CAD build for the part. Positions are in the model's coordinates, mm. Face numbers are marked on the shaded views. A direction names the side the tool comes from. Give positions to 0.01 mm unless a question says otherwise; leave off trailing zeros. Order: outer loops, then holes, each group sorted by start corner. A loop starts at its lowest first (then second) coordinate and runs counter-clockwise, first axis right, second up. Notation, with made-up numbers: M 71,24 L 110,24 A17 ccw 110,31 Z; hole C 19,-6 d9. An arc over 180 degrees is marked long. Put each result on its own line as item: value. Start each with the question number.
1) Drill centre lines: line 1 (Y direction, x = 0, z = -19.5); line 2 (X direction, y = 5, z = -25); line 3 (Z direction, x = 0.5, y = -172.5). Where is each one in solid material? Low to high. Write a range as [from, to].
2) Pin check, flat tips, straight feed: pin 1 (10 mm diameter, centred on x = 2.5, z = -7, fed in from +Y); pin 2 (4 mm diameter, centred on x = 2, y = -141, fed in from -Z). Stop position of each tip, or through.
3) Cut at C-C (z = 18). Write the cut outline in (x, y), and give its area (3 significant figures).
4) Cut at B-B (x = -11). Write the cut outline in (y, z).
5) Cut at A-A (z = -30). Write the cut outline in (x, y).
6) Cut at D-D (y = -171). Write the cut outline in (x, z).
7) Tool access for the marked faces 1 and 2: list every direction of +Z, -Z, +X, -X, +Y, -Y with a clear straight run to the whole face (end or side of a thin tool).
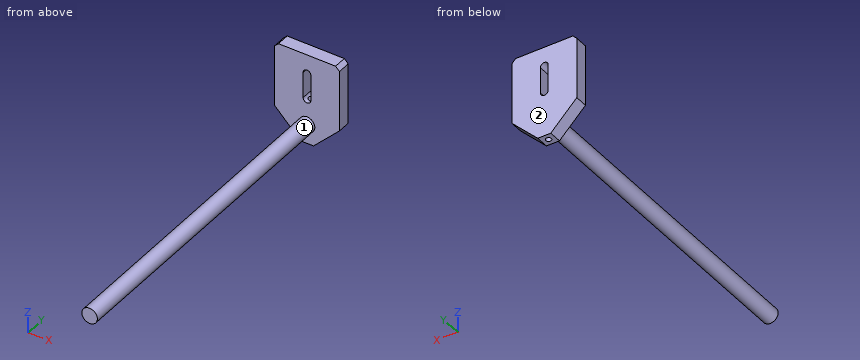
```python
from build123d import *

# Parameters (mm, degrees)
BOSS_EXTRUDE1_DEPTH   = 10
SKETCH2_R             = 6
BOSS_EXTRUDE2_DEPTH   = 260
CUT_EXTRUDE1_DEPTH    = 256.244980362
M5_TAPPED_HOLE1_D     = 4.2
M5_TAPPED_HOLE1_DEPTH = 36.9
M5_TAPPED_HOLE1_TIP   = 1.2618073
CHAMFER1_SIZE         = 3


with BuildPart() as part:
    # Sketch1 → Boss-Extrude1 (new body)
    with BuildSketch(Plane(origin=(0, 0, 0), x_dir=(1, 0, 0), z_dir=(0, 1, 0))):
        Polygon((-25, 25), (-5, 45), (5, 45), (25, 25), (25, -25), (-25, -25), align=None)
    extrude(amount=BOSS_EXTRUDE1_DEPTH)

    # Sketch2 → Boss-Extrude2 (add)
    with BuildSketch(Plane.XZ.offset(-10)):
        with Locations(Location((0, -30, 0), (0, 0, 90))):
            Circle(SKETCH2_R)
    extrude(amount=BOSS_EXTRUDE2_DEPTH)

    # Sketch3 → Cut-Extrude1 (cut, through all)
    with BuildSketch(Plane.XZ):
        with BuildLine():
            Line((-3, -10), (-3, 10))
            ThreePointArc((-3, 10), (0, 13), (3, 10))
            Line((3, 10), (3, -10))
            ThreePointArc((3, -10), (0, -13), (-3, -10))
        make_face()
    extrude(amount=-CUT_EXTRUDE1_DEPTH, mode=Mode.SUBTRACT)

    # M5 Tapped Hole1
    with Locations(Plane(origin=(0, 0, -45), x_dir=(-1, 0, 0), z_dir=(0, 0, -1))):
        with Locations((0, 5)):
            Hole(M5_TAPPED_HOLE1_D / 2, depth=M5_TAPPED_HOLE1_DEPTH)
            with Locations((0, 0, -(M5_TAPPED_HOLE1_DEPTH + M5_TAPPED_HOLE1_TIP / 2))):  # 118° drill point
                Cone(0, M5_TAPPED_HOLE1_D / 2, M5_TAPPED_HOLE1_TIP, mode=Mode.SUBTRACT)

    # Chamfer1
    chamfer1_edges = [part.edges().sort_by_distance(p)[0] for p in [
        (25, 5, 25),
        (-25, 5, 25),
    ]]
    chamfer(chamfer1_edges, length=CHAMFER1_SIZE)


solid = part.part
```
Solution:
1. line 1: [0, 2.9], [7.1, 10]
1. line 2: [-25, -2.1], [2.1, 25]
1. line 3: [-35.98, -24.02]
2. pin 1: y = 10
2. pin 2: z = -36
3. outline: M -25,0 L 25,0 L 25,10 L -25,10 Z
3. area: 500 mm²
4. outline: M 0,-39 L 10,-39 L 10,25 L 0,25 Z
5. outline: M -20,0 L -6,0 L -6,-250 L 6,-250 L 6,0 L 20,0 L 20,10 L -20,10 Z; hole C 0,5 d4.2
6. outline: C 0,-30 d12
7. face 1: -Y
7. face 2: +Z, -Z, +X, -X, +Y
